from build123d import *

# Parameters (mm, degrees)
SKETCH1_W           = 20
SKETCH1_H           = 30
BOSS_EXTRUDE1_DEPTH = 3
SKETCH2_R           = 2.3
CUT_EXTRUDE1_DEPTH  = 3
FILLET1_R           = 3


with BuildPart() as part:
    # Sketch1 → Boss-Extrude1 (new body)
    with BuildSketch(Plane.XY):
        Rectangle(SKETCH1_W, SKETCH1_H)
    extrude(amount=BOSS_EXTRUDE1_DEPTH)

    # Sketch2 → Cut-Extrude1 (cut)
    with BuildSketch(Plane.XY.offset(3)):
        with Locations((-5.05, 10)):
            Circle(SKETCH2_R)
        with Locations((5.05, 10)):
            Circle(SKETCH2_R)
        with Locations((-5.05, -10)):
            Circle(SKETCH2_R)
        with Locations((5.05, -10)):
            Circle(SKETCH2_R)
    extrude(amount=-CUT_EXTRUDE1_DEPTH, mode=Mode.SUBTRACT)

    # Fillet1
    fillet1_edges = [part.edges().sort_by_distance(p)[0] for p in [
        (10, -15, 1.5),
        (-10, -15, 1.5),
        (-10, 15, 1.5),
        (10, 15, 1.5),
    ]]
    fillet(fillet1_edges, radius=FILLET1_R)


solid = part.part
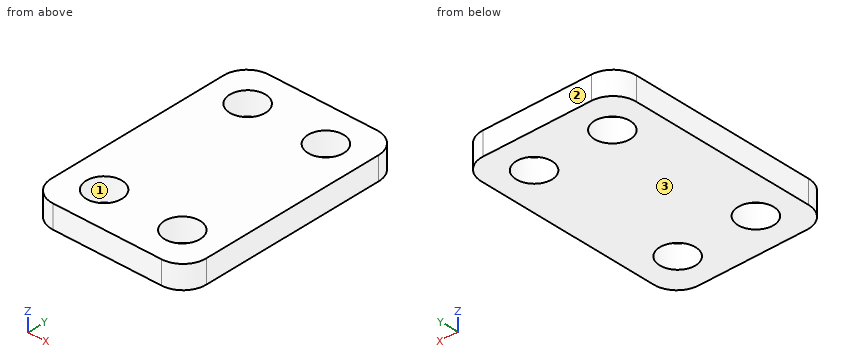
Verification items for the finished model (mm, model axes). Face numbers are marked on the shaded views. Give positions to 0.01 mm unless a question says otherwise; leave off trailing zeros. Write each loop counter-clockwise with the first axis right and the second up, starting at its lowest first coordinate (ties: lowest second). Pieces come first, ordered by that corner, then holes.
(1) Mould release check, pull along Y, two halves, no side actions. Record for the marked faces 1, 2 and 3: +Y half, -Y half, draft (parallel to the pull), parting line (faces both ways), or undercut.
(2) Material ranges on line 1 (Y direction, x = -5.05, z = 2.3); line 2 (X direction, y = -8.75, z = 0.5); line 3 (X direction, y = 9.5, z = 0.35) (3 decimals), recorded low to high.
(3) Gauge pin test, flat end, axial feed: pin 1 (3.5 mm diameter, centred on x = 5.05, y = -10, fed in from +Z). Record the tip position at first contact, or that the pin passes through.
(4) Cross-section at B-B (y = -10). Enter the section's corners in (x, z), plus the area to 3 significant figures.
(5) Cross-section at D-D (y = -13). Enter the section's corners in (x, z).
(6) Cross-section at A-A (x = 5.05). Enter the section's corners in (y, z).
(7) Cross-section at C-C (z = 2.1). Enter the section's corners in (x, y).
Worked out:
1. face 1: undercut
1. face 2: +Y half
1. face 3: draft
2. line 1: y = -15 to -12.3, -7.7 to 7.7, 12.3 to 15
2. line 2: x = -10 to -6.98, -3.12 to 3.12, 6.98 to 10
2. line 3: x = -10 to -7.295, -2.805 to 2.805, 7.295 to 10
3. pin 1: passes through
4. outline: (-10, 0) - (-7.35, 0) - (-7.35, 3) - (-10, 3) - close; (-2.75, 0) - (2.75, 0) - (2.75, 3) - (-2.75, 3) - close; (7.35, 0) - (10, 0) - (10, 3) - (7.35, 3) - close
4. area: 32.4 mm2
5. outline: (-9.83, 0) - (9.83, 0) - (9.83, 3) - (-9.83, 3) - close
6. outline: (-15, 0) - (-12.3, 0) - (-12.3, 3) - (-15, 3) - close; (-7.7, 0) - (7.7, 0) - (7.7, 3) - (-7.7, 3) - close; (12.3, 0) - (15, 0) - (15, 3) - (12.3, 3) - close
7. outline: (-10, -12) arc R3 ccw to (-7, -15) - (7, -15) arc R3 ccw to (10, -12) - (10, 12) arc R3 ccw to (7, 15) - (-7, 15) arc R3 ccw to (-10, 12) - close; hole circle Ø4.6 at (-5.05, -10); hole circle Ø4.6 at (-5.05, 10); hole circle Ø4.6 at (5.05, -10); hole circle Ø4.6 at (5.05, 10)
